Geometry: final body of the model. Coordinates: model frame, mm. Give positions to 0.01 mm unless a question says otherwise; leave off trailing zeros. Write each loop counter-clockwise with the first axis right and the second up, starting at its lowest first coordinate (ties: lowest second). Pieces come first, ordered by that corner, then holes. Notation, with made-up numbers: (89.25, 9) -> (139.25, 9) arc R11 cw to (139.25, 25) -> close; hole circle Ø3 at (33.25, -2). An arc over 180 degrees is marked (long way). Answer as a JSON object with one key per item and string values.
from build123d import *

# Parameters (mm, degrees)
SKETCH_1_R      = 25
EXTRUDE_1_DEPTH = 20
SKETCH_2_W      = 100
SKETCH_2_H      = 300
SKETCH_2_R      = 20
EXTRUDE_2_DEPTH = 20
FILLET_1_R      = 20


with BuildPart() as part:
    # 草图1 → 凸台-拉伸1 (new body)
    with BuildSketch(Plane.XY):
        Circle(SKETCH_1_R)
    extrude(amount=EXTRUDE_1_DEPTH)

    # 草图2 → 凸台-拉伸2 (add)
    with BuildSketch(Plane(origin=(0, 0, 0), x_dir=(-1, 0, 0), z_dir=(0, 0, -1))):
        with Locations((0, 100)):
            Rectangle(SKETCH_2_W, SKETCH_2_H)
        with Locations((0, 200)):
            Circle(SKETCH_2_R, mode=Mode.SUBTRACT)
    extrude(amount=EXTRUDE_2_DEPTH)

    # 圆角1
    fillet_1_edges = [part.edges().sort_by_distance(p)[0] for p in [
        (-50, 250, -10),
        (50, 250, -10),
    ]]
    fillet(fillet_1_edges, radius=FILLET_1_R)


solid = part.part
Q1. Material intervals for L1, parallel to Y at x = 0, z = -6.75; L2, parallel to Z at x = 22, y = 135.5; L3, parallel to X at y = 0.5, z = 17.5 (3 decimals), sorted ascending. Write a range as from..to.
Values:
{"L1": "-50..180, 220..250", "L2": "-20..0", "L3": "-24.995..24.995"}
Q2. Cut plane C-C (z = -4.5). Return the cut outline in (x, y).
Values:
{"outline": "(-50, -50) -> (50, -50) -> (50, 230) arc R20 ccw to (30, 250) -> (-30, 250) arc R20 ccw to (-50, 230) -> close; hole circle Ø40 at (0, 200)"}
Q3. First-contact query: P1, Ø3, axis at x = -33.5, y = 140, coming from the +Z side. Flat tip, straight axial feed; report the tip coordinate or a pass-through.
Values:
{"P1": "z = 0"}
Q4. Cut plane A-A (y = 200). Return the cut outline in (x, z).
Values:
{"outline": "(-50, -20) -> (-20, -20) -> (-20, 0) -> (-50, 0) -> close; (20, -20) -> (50, -20) -> (50, 0) -> (20, 0) -> close"}
Q5. Cut plane D-D (y = 0). Return the cut outline in (x, z).
Values:
{"outline": "(-50, -20) -> (50, -20) -> (50, 0) -> (25, 0) -> (25, 20) -> (-25, 20) -> (-25, 0) -> (-50, 0) -> close"}
Q6. Mould query, pull axis Y, two halves, no side actions, for faces 1 (the flat face through (1, -50, -10)), 2 (the flat face through (0, 250, -10)), 3 (the cylindrical face through (23.846, 7.509, 9.86)), 4 (the cylindrical face through (2.6, 219.83, -9.86)). Classes: pulls with the +Y half, pulls with the -Y half, needs draft (parallel to the pull), parting line crosses it, or undercut.
Values:
{"face 1": "pulls with the -Y half", "face 2": "pulls with the +Y half", "face 3": "parting line crosses it", "face 4": "undercut"}
Q7. Cut plane B-B (x = 0). Return the cut outline in (y, z), and give its area (3 significant figures).
Values:
{"outline": "(-50, -20) -> (180, -20) -> (180, 0) -> (25, 0) -> (25, 20) -> (-25, 20) -> (-25, 0) -> (-50, 0) -> close; (220, -20) -> (250, -20) -> (250, 0) -> (220, 0) -> close", "area": "6,200 mm²"}
